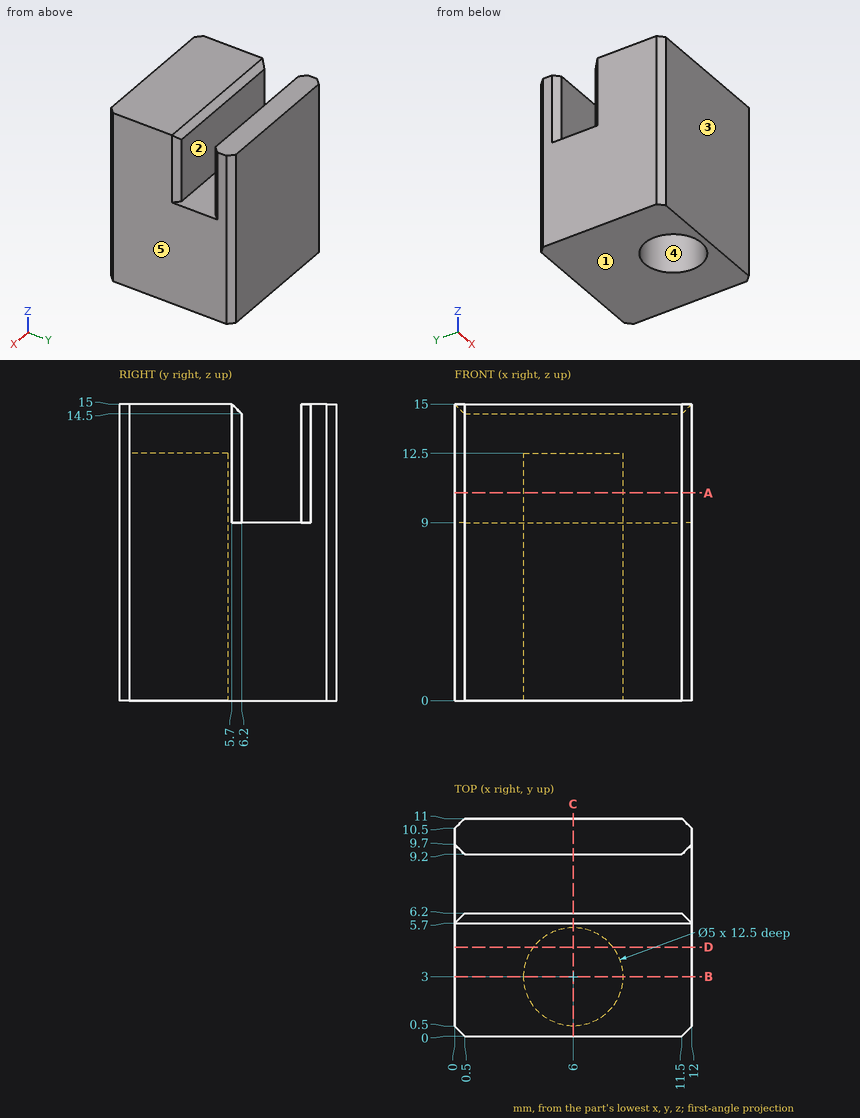
Job drawing, mm, ordinate dimensions from the low corner. One solid piece. A direction names the side the tool comes from. Coordinates: 2 decimals unless noted, no trailing zeros. Write each loop counter-clockwise with the first axis right and the second up, starting at its lowest first coordinate (ties: lowest second). Pieces come first, ordered by that corner, then holes. Notation, with made-up numbers: (30.25, -21.5) - (36.25, -21.5) arc R20 ccw to (36.25, 1.5) - close; hole circle Ø5 at (-2, 87.25). An arc over 180 degrees is marked (long way). Use a Markdown table: item, result. Add a question column.
Item 1: Band-saw the part on B-B, the plane y = 3. Give the cut face in (x, z).
Item 2: 3-axis set-ups, long thin cutter, end or side, ignore diameter. For the marked faces 1 and 2: which of +Z, -Z, +X, -X, +Y, -Y reach the whole face in a straight line?
Item 3: Band-saw the part on C-C, the plane x = 6. Give the cut face in (y, z).
Item 4: Band-saw the part on D-D, the plane y = 4.5. Give the cut face in (x, z).
Item 5: Flat gauge pins, fed straight in: pin 1 (1.2 mm diameter, centred on x = 6, y = 7, fed in from +Z); pin 2 (1.5 mm diameter, centred on x = 6.5, y = 2, fed in from -Z); pin 3 (1 mm diameter, centred on x = 9.5, y = 6.5, fed in from +Z). Where does each tip first touch, or does it go through?
Item 6: Mould opens along X. For the marked faces 3, 4 and 5 say: pulls with the +X half, pulls with the -X half, needs draft (parallel to the pull), parting line crosses it, or undercut.
Item 7: Drill centre lines: L1, parallel to Y at x = 6, z = 9.25; L2, parallel to Y at x = 6, z = 4; L3, parallel to Y at x = 5.5, z = 9.25. Where is each one in solid material? Low to high. Write a range as from..to.
Item 8: Band-saw the part on A-A, the plane z = 10.5. Give the cut face in (x, y).
Numbers:
| question | item | result |
|---|---|---|
| 1 | outline | (0, 0) - (3.5, 0) - (3.5, 12.5) - (8.5, 12.5) - (8.5, 0) - (12, 0) - (12, 15) - (0, 15) - close |
| 2 | face 1 | -Z, +X, -X, +Y, -Y |
| 2 | face 2 | +Z, +X, -X |
| 3 | outline | (0, 0) - (0.5, 0) - (0.5, 12.5) - (5.5, 12.5) - (5.5, 0) - (11, 0) - (11, 15) - (9.2, 15) - (9.2, 9) - (6.2, 9) - (6.2, 14.5) - (5.7, 15) - (0, 15) - close |
| 4 | outline | (0, 0) - (4, 0) - (4, 12.5) - (8, 12.5) - (8, 0) - (12, 0) - (12, 15) - (0, 15) - close |
| 5 | pin 1 | z = 9 |
| 5 | pin 2 | z = 12.5 |
| 5 | pin 3 | z = 14.7 |
| 6 | face 3 | needs draft |
| 6 | face 4 | undercut |
| 6 | face 5 | pulls with the +X half |
| 7 | L1 | 0..0.5, 5.5..6.2, 9.2..11 |
| 7 | L2 | 0..0.5, 5.5..11 |
| 7 | L3 | 0..0.55, 5.45..6.2, 9.2..11 |
| 8 | outline | (0, 0.5) - (0.5, 0) - (11.5, 0) - (12, 0.5) - (12, 5.7) - (11.5, 6.2) - (0.5, 6.2) - (0, 5.7) - close; (0, 9.7) - (0.5, 9.2) - (11.5, 9.2) - (12, 9.7) - (12, 10.5) - (11.5, 11) - (0.5, 11) - (0, 10.5) - close; hole circle Ø5 at (6, 3) |
